```python
from build123d import *

# Parameters (mm, degrees)
SKETCH1_R           = 19
SKETCH1_R_2         = 7
BOSS_EXTRUDE1_DEPTH = 0.3


with BuildPart() as part:
    # Sketch1 → Boss-Extrude1 (new, symmetric)
    with BuildSketch(Plane(origin=(0, 0, 0), x_dir=(1, 0, 0), z_dir=(0, 1, 0))):
        with BuildLine():
            Line((-130, 83), (-130, -83))
            ThreePointArc((-130, -83), (-128.535533906, -86.535533906), (-125, -88))
            Line((-125, -88), (180, -88))
            ThreePointArc((180, -88), (183.535533906, -86.535533906), (185, -83))
            Line((185, -83), (185, 83))
            ThreePointArc((185, 83), (183.535533906, 86.535533906), (180, 88))
            Line((180, 88), (-125, 88))
            ThreePointArc((-125, 88), (-128.535533906, 86.535533906), (-130, 83))
        make_face()
        with Locations(Location((0, 34, 0), (0, 0, 270))):
            Circle(SKETCH1_R, mode=Mode.SUBTRACT)
        with Locations(Location((0, -34, 0), (0, 0, 270))):
            Circle(SKETCH1_R, mode=Mode.SUBTRACT)
        with Locations(Location((-95, -15, 0), (0, 0, 270))):
            Circle(SKETCH1_R_2, mode=Mode.SUBTRACT)
    extrude(amount=BOSS_EXTRUDE1_DEPTH, both=True)


solid = part.part
```
The listing builds one solid part. Answer for the finished solid, in the listing's coordinates (mm). Give positions to 0.01 mm unless a question says otherwise; leave off trailing zeros. Loops run counter-clockwise (first coordinate to the right, second up) from the corner with the lowest first, then second, coordinate; pieces in that order, holes last. Notation, with made-up numbers: (75, 75.5) - (104, 75.5) arc R22 ccw to (104, 91.5) - close; hole circle Ø11 at (73.25, 5). An arc over 180 degrees is marked (long way). Answer as CSV lines item,"result". Start each with the question number.
Item 1: A cutting plane is placed at C-C on y = -0.05. Determine the outline of the cut face in (x, z), then the cut area to 3 significant figures.
Item 2: A cutting plane is placed at B-B on x = 0. Determine the outline of the cut face in (y, z), then the cut area to 3 significant figures.
Item 3: A cutting plane is placed at A-A on z = 34. Determine the outline of the cut face in (x, y), then the cut area to 3 significant figures.
Item 4: Find the intervals of material crossed by line 1 (X direction, y = 0, z = -34); line 2 (X direction, y = 0.05, z = 51.5), in increasing order. Write a range as from..to.
Item 5: The mould has two halves that part along Z. Classify faces 1 (the face through (25, -0.3, -1)), 2 (the face through (-88.06, 0, 14.09)): +Z half, -Z half, draft (parallel to the pull), parting line (faces both ways), or undercut.
Item 6: A cutting plane is placed at D-D on z = -20. Determine the outline of the cut face in (x, y).
Found:
1,outline,"(-130, -83) arc R5 ccw to (-125, -88) - (180, -88) arc R5 ccw to (185, -83) - (185, 83) arc R5 ccw to (180, 88) - (-125, 88) arc R5 ccw to (-130, 83) - close; hole circle Ø14 at (-95, 15); hole circle Ø38 at (0, -34); hole circle Ø38 at (0, 34)"
1,area,"53,000 mm^2"
2,outline,"(-0.3, -88) - (0.3, -88) - (0.3, -53) - (-0.3, -53) - close; (-0.3, -15) - (0.3, -15) - (0.3, 15) - (-0.3, 15) - close; (-0.3, 53) - (0.3, 53) - (0.3, 88) - (-0.3, 88) - close"
2,area,"60.0 mm^2"
3,outline,"(-130, -0.3) - (-19, -0.3) - (-19, 0.3) - (-130, 0.3) - close; (19, -0.3) - (185, -0.3) - (185, 0.3) - (19, 0.3) - close"
3,area,"166 mm^2"
4,line 1,"x = -130..-19, 19..185"
4,line 2,"x = -130..-7.4, 7.4..185"
5,face 1,"draft"
5,face 2,"undercut"
6,outline,"(-130, -0.3) - (-12.85, -0.3) - (-12.85, 0.3) - (-130, 0.3) - close; (12.85, -0.3) - (185, -0.3) - (185, 0.3) - (12.85, 0.3) - close"
